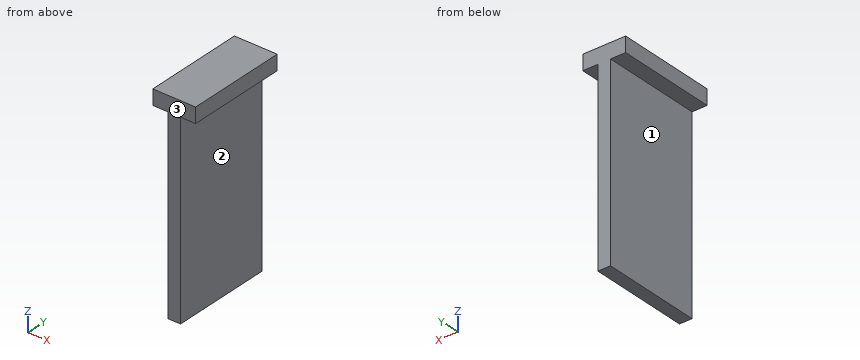
from build123d import *

# Parameters (mm, degrees)
SKETCH_1_W      = 150
SKETCH_1_H      = 80
EXTRUDE_1_DEPTH = 5
SKETCH_2_W      = 22
SKETCH_2_H      = 80
EXTRUDE_2_DEPTH = 12


with BuildPart() as part:
    # 草图1 → 凸台-拉伸1 (new, symmetric)
    with BuildSketch(Plane(origin=(0, 0, 0), x_dir=(0, 0, -1), z_dir=(1, 0, 0))):
        Rectangle(SKETCH_1_W, SKETCH_1_H)
    extrude(amount=EXTRUDE_1_DEPTH, both=True)

    # 草图2 → 凸台-拉伸2 (add)
    with BuildSketch(Plane.XY.offset(75)):
        with Locations((6, 0)):
            Rectangle(SKETCH_2_W, SKETCH_2_H)
    extrude_2 = extrude(amount=EXTRUDE_2_DEPTH)

    # 镜向1: 凸台-拉伸2 across plane
    add(extrude_2.mirror(Plane(origin=(0, 0, 0), x_dir=(0, 0, 1), z_dir=(1, 0, 0))))


solid = part.part
Check sheet for the modelled part. Datum: model origin and axes. Units: mm. Face numbers are marked on the shaded views. A direction names the side the tool comes from. Round coordinates to 2 decimals unless told otherwise and drop trailing zeros. Order: outer loops, then holes, each group sorted by start corner. A loop starts at its lowest first (then second) coordinate and runs counter-clockwise, first axis right, second up.
Q1. Cross-section at C-C, the plane x = 14. Enter the section's corners in (y, z).
Filled sheet:
outline: (-40, 75) - (40, 75) - (40, 87) - (-40, 87) - close
Q2. Cross-section at A-A, the plane y = 10. Enter the section's corners in (x, z).
Filled sheet:
outline: (-17, 75) - (-5, 75) - (-5, -75) - (5, -75) - (5, 75) - (17, 75) - (17, 87) - (-17, 87) - close
Q3. Depth check by flat-ended pin: P1, Ø8, axis at x = -11.5, y = 26.5, coming from the -Z side; P2, Ø10, axis at y = 9.5, z = 18, coming from the -X side; P3, Ø1.5, axis at y = -16.5, z = 36, coming from the +X side. Enter the tip coordinate at first touch or a pass-through.
Filled sheet:
P1: stops at z = 75
P2: stops at x = -5
P3: stops at x = 5
Q4. Set-up check for the marked faces 1, 2 and 3: record each of +Z, -Z, +X, -X, +Y, -Y from which the full face is reachable in a straight line by a thin tool's end or side.
Filled sheet:
face 1: -Z, -X, +Y, -Y
face 2: -Z, +X, +Y, -Y
face 3: +Z, -Z, +X, -X, -Y
Q5. Scan lines: L1, parallel to Z at x = 9, y = -35; L2, parallel to X at y = 18.5, z = -59.5. Record each from-to range of solid material in increasing order.
Filled sheet:
L1: z = 75 to 87
L2: x = -5 to 5
Q6. Cross-section at B-B, the plane z = -59. Enter the section's corners in (x, y).
Filled sheet:
outline: (-5, -40) - (5, -40) - (5, 40) - (-5, 40) - close
